Read the model definition and answer for the solid it produces. Units are mm, in the model's axes. Face numbers are marked on the shaded views. A direction names the side the tool comes from. Coordinates: 2 decimals unless noted, no trailing zeros. Order: outer loops, then holes, each group sorted by start corner. A loop starts at its lowest first (then second) coordinate and runs counter-clockwise, first axis right, second up.
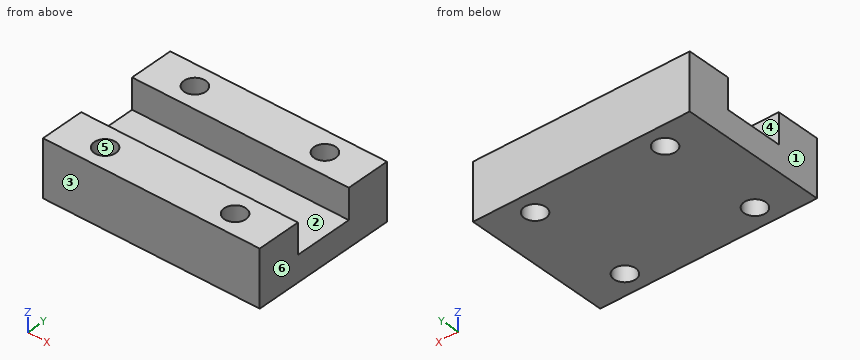
```python
from build123d import *

# Parameters (mm, degrees)
SKETCH_1_W          = 25
SKETCH_1_H          = 17
EXTRUDE_1_DEPTH     = 6.5
CUT_EXTRUDE_1_REACH = 30.286
SKETCH_2_W          = 3.5
SKETCH_2_H          = 6.8
CUT_EXTRUDE_2_REACH = 20.562
SKETCH_3_R          = 1.25


with BuildPart() as part:
    # 草图1 → 凸台-拉伸1 (new body)
    with BuildSketch(Plane.XY):
        with Locations((-0.517429194, 3.026143791)):
            Rectangle(SKETCH_1_W, SKETCH_1_H)
    extrude(amount=EXTRUDE_1_DEPTH)

    # 草图2 → 切除-拉伸1 (cut, up to next)
    with BuildSketch(Plane(origin=(11.982570806, 0, 0), x_dir=(0, 0, -1), z_dir=(1, 0, 0)), mode=Mode.PRIVATE) as cut_extrude_1_sk1:
        with Locations((-4.75, 3.026143791)):
            Rectangle(SKETCH_2_W, SKETCH_2_H)
    cut_extrude_1_tool1 = extrude(cut_extrude_1_sk1.sketch, amount=-CUT_EXTRUDE_1_REACH, mode=Mode.PRIVATE) & part.part
    add(cut_extrude_1_tool1.solids().sort_by_distance((11.982571, 3.026144, 4.75))[0], mode=Mode.SUBTRACT)

    # 草图3 → 切除-拉伸2 (cut, up to next)
    with BuildSketch(Plane.XY.offset(6.5), mode=Mode.PRIVATE) as cut_extrude_2_sk1:
        with Locations((-8.017429194, 9.026143791)):
            Circle(SKETCH_3_R)
    cut_extrude_2_tool1 = extrude(cut_extrude_2_sk1.sketch, amount=-CUT_EXTRUDE_2_REACH, mode=Mode.PRIVATE) & part.part
    # 草图3 → 切除-拉伸2 (cut, up to next)
    with BuildSketch(Plane.XY.offset(6.5), mode=Mode.PRIVATE) as cut_extrude_2_sk2:
        with Locations((6.982570806, 9.026143791)):
            Circle(SKETCH_3_R)
    cut_extrude_2_tool2 = extrude(cut_extrude_2_sk2.sketch, amount=-CUT_EXTRUDE_2_REACH, mode=Mode.PRIVATE) & part.part
    # 草图3 → 切除-拉伸2 (cut, up to next)
    with BuildSketch(Plane.XY.offset(6.5), mode=Mode.PRIVATE) as cut_extrude_2_sk3:
        with Locations((-8.017429194, -2.973856209)):
            Circle(SKETCH_3_R)
    cut_extrude_2_tool3 = extrude(cut_extrude_2_sk3.sketch, amount=-CUT_EXTRUDE_2_REACH, mode=Mode.PRIVATE) & part.part
    # 草图3 → 切除-拉伸2 (cut, up to next)
    with BuildSketch(Plane.XY.offset(6.5), mode=Mode.PRIVATE) as cut_extrude_2_sk4:
        with Locations((6.982570806, -2.973856209)):
            Circle(SKETCH_3_R)
    cut_extrude_2_tool4 = extrude(cut_extrude_2_sk4.sketch, amount=-CUT_EXTRUDE_2_REACH, mode=Mode.PRIVATE) & part.part
    add(cut_extrude_2_tool1.solids().sort_by_distance((-8.017429, 9.026144, 6.5))[0], mode=Mode.SUBTRACT)
    add(cut_extrude_2_tool2.solids().sort_by_distance((6.982571, 9.026144, 6.5))[0], mode=Mode.SUBTRACT)
    add(cut_extrude_2_tool3.solids().sort_by_distance((-8.017429, -2.973856, 6.5))[0], mode=Mode.SUBTRACT)
    add(cut_extrude_2_tool4.solids().sort_by_distance((6.982571, -2.973856, 6.5))[0], mode=Mode.SUBTRACT)


solid = part.part
```
1) Flat-ended cylindrical pins translate along their axes: pin 1 Ø3.5 at (x, y) = (-4.5, 2) entering from +Z; pin 2 Ø2 at (x, y) = (-8.02, -2.97) entering from -Z. Find the tip coordinate at first contact, or state that the pin passes through.
A:
pin 1: stops at z = 3
pin 2: passes through
2) Determine the mould class of the marked faces 3, 4, 5 and 6 for opening direction Y: pulls with the +Y half, pulls with the -Y half, needs draft (parallel to the pull), parting line crosses it, or undercut.
A:
face 3: pulls with the -Y half
face 4: undercut
face 5: undercut
face 6: needs draft
3) A cutting plane is placed at D-D, the plane y = -2.5. Determine the outline of the cut face in (x, z), and give its area (3 significant figures).
A:
outline: (-13.02, 0) - (-9.17, 0) - (-9.17, 6.5) - (-13.02, 6.5) - close; (-6.86, 0) - (5.83, 0) - (5.83, 6.5) - (-6.86, 6.5) - close; (8.14, 0) - (11.98, 0) - (11.98, 6.5) - (8.14, 6.5) - close
area: 132 mm2
4) A cutting plane is placed at C-C, the plane x = -8. Determine the outline of the cut face in (y, z).
A:
outline: (-5.47, 0) - (-4.22, 0) - (-4.22, 6.5) - (-5.47, 6.5) - close; (-1.72, 0) - (7.78, 0) - (7.78, 6.5) - (6.43, 6.5) - (6.43, 3) - (-0.37, 3) - (-0.37, 6.5) - (-1.72, 6.5) - close; (10.28, 0) - (11.53, 0) - (11.53, 6.5) - (10.28, 6.5) - close
5) Straight lines are drawn through the part: line 1 (Y direction, x = 2.5, z = 3.5); line 2 (X direction, y = -4, z = 3.25); line 3 (Y direction, x = -7, z = 1.75). For each, find the intervals that lie inside material, in ascending order.
A:
line 1: y = -5.47 to -0.37, 6.43 to 11.53
line 2: x = -13.02 to -8.73, -7.3 to 6.27, 7.7 to 11.98
line 3: y = -5.47 to -3.7, -2.25 to 8.3, 9.75 to 11.53
6) A cutting plane is placed at B-B, the plane x = -1.5. Determine the outline of the cut face in (y, z).
A:
outline: (-5.47, 0) - (11.53, 0) - (11.53, 6.5) - (6.43, 6.5) - (6.43, 3) - (-0.37, 3) - (-0.37, 6.5) - (-5.47, 6.5) - close
7) A cutting plane is placed at A-A, the plane z = 5.5. Determine the outline of the cut face in (x, y).
A:
outline: (-13.02, -5.47) - (11.98, -5.47) - (11.98, -0.37) - (-13.02, -0.37) - close; (-13.02, 6.43) - (11.98, 6.43) - (11.98, 11.53) - (-13.02, 11.53) - close; hole circle Ø2.5 at (-8.02, -2.97); hole circle Ø2.5 at (-8.02, 9.03); hole circle Ø2.5 at (6.98, -2.97); hole circle Ø2.5 at (6.98, 9.03)
8) Which of the six approach directions +Z, -Z, +X, -X, +Y, -Y give full straight-line access (tool end or side, diameter ignored) to the marked faces 1 and 2?
A:
face 1: +Z, -Z, -X, +Y, -Y
face 2: +Z, +X, -X
